Could you check a few things on this model? Use its own coordinates, in mm. Face numbers are marked on the shaded views. Round coordinates to 2 decimals unless told otherwise and drop trailing zeros. Loops run counter-clockwise (first coordinate to the right, second up) from the corner with the lowest first, then second, coordinate; pieces in that order, holes last. Notation, with made-up numbers: (85, -35.75) - (127, -35.75) arc R12 ccw to (127, -29.75) - close; hole circle Ø10 at (87.25, 57.25). An arc over 180 degrees is marked (long way). Answer as CSV lines item,"result". Start each with the question number.
1) I'm going to push flat-ended pins straight in: pin 1 Ø6 at (x, y) = (-373, 93) entering from +Z; pin 2 Ø2 at (x, y) = (-18.5, -324) entering from +Z. Where does each tip first touch, or does it pass through?
2) Please list where these lines run through material, in increasing order: line 1 along X through (y, z) = (324.2, 670); line 2 along Z through (x, y) = (488.8, 295); line 3 along Z through (x, y) = (474, -324.05).
3) Suppose I cut it at A-A, the plane z = 288. Write out the boundary of the cut face in (x, y).
4) Suppose I cut it at C-C, the plane x = -194. Write out the boundary of the cut face in (y, z), then the cut area to 3 significant figures.
5) We'd pull the mould along X, two halves only. Please class the marked faces 1, 2, 3 and 4: pulls with the +X half, pulls with the -X half, needs draft (parallel to the pull), parting line crosses it, or undercut.
6) Suppose I cut it at B-B, the plane y = -149. Write out the boundary of the cut face in (x, z).
```python
from build123d import *

# Parameters (mm, degrees)
EXTRUDE_1_DEPTH          = 325
EXTRUDE_2_DEPTH          = 2
EXTRUDE_3_DEPTH          = 2
SKETCH_5_W               = 30
SKETCH_5_H               = 650
EXTRUDE_4_DEPTH          = 2
SKETCH_6_R               = 4.5
CUT_EXTRUDE_1_DEPTH      = 10
CUT_EXTRUDE_2_DEPTH      = 1140
CUT_EXTRUDE_2_DEPTH_BACK = 345
SKETCH_7_R               = 4.5
SKETCH_8_R               = 4.5
CUT_EXTRUDE_3_DEPTH      = 10


with BuildPart() as part:
    # 草图1 → 凸台-拉伸1 (new, symmetric)
    with BuildSketch(Plane(origin=(0, 0, 0), x_dir=(1, 0, 0), z_dir=(0, 1, 0))):
        Polygon((-490, 700), (490, 700), (490, -700), (488, -700), (488, 698), (-488, 698), (-488, -700), (-490, -700), align=None)
    extrude(amount=EXTRUDE_1_DEPTH, both=True)

    # 草图2 → 凸台-拉伸2 (add)
    with BuildSketch(Plane(origin=(0, 325, 0), x_dir=(1, 0, 0), z_dir=(0, 1, 0))):
        Polygon((-490, 700), (-490, -700), (-460, -700), (-460, 670), (460, 670), (460, -700), (490, -700), (490, 700), align=None)
    extrude(amount=-EXTRUDE_2_DEPTH)

    # 草图3 → 凸台-拉伸3 (add)
    with BuildSketch(Plane.XZ.offset(325)):
        Polygon((490, -700), (490, 700), (460, 700), (460, -670), (-460, -670), (-460, 700), (-490, 700), (-490, -700), align=None)
    extrude(amount=-EXTRUDE_3_DEPTH)

    # 草图5 → 凸台-拉伸4 (add)
    with BuildSketch(Plane.XY.offset(700)):
        with Locations((-475, 0)):
            Rectangle(SKETCH_5_W, SKETCH_5_H)
    extrude(amount=-EXTRUDE_4_DEPTH)

    # 草图6 → 切除-拉伸1 (cut)
    with BuildSketch(Plane(origin=(0, 0, 698), x_dir=(-1, 0, 0), z_dir=(0, 0, -1))):
        with Locations((474, -246)):
            Circle(SKETCH_6_R)
        with Locations((474, -186)):
            Circle(SKETCH_6_R)
        with Locations((474, 295)):
            Circle(SKETCH_6_R)
        with Locations((474, 57)):
            Circle(SKETCH_6_R)
        with Locations((474, -23)):
            Circle(SKETCH_6_R)
        with Locations((474, -123)):
            Circle(SKETCH_6_R)
    extrude(amount=-CUT_EXTRUDE_1_DEPTH, mode=Mode.SUBTRACT)

    # 草图7 → 切除-拉伸2 (cut, two sides: drawn at the far end of the back side and taken through both)
    with BuildSketch(Plane.XZ.offset(-323).offset(-CUT_EXTRUDE_2_DEPTH_BACK)):
        with Locations(Location((-474, 670, 0), (0, 0, 90))):
            Circle(SKETCH_7_R)
        with Locations(Location((-474, 0, 0), (0, 0, 90))):
            Circle(SKETCH_7_R)
        with Locations(Location((-474, -684, 0), (0, 0, 90))):
            Circle(SKETCH_7_R)
        with Locations(Location((474, -684, 0), (0, 0, 90))):
            Circle(SKETCH_7_R)
        with Locations(Location((0, -684, 0), (0, 0, 90))):
            Circle(SKETCH_7_R)
        with Locations(Location((474, 0, 0), (0, 0, 90))):
            Circle(SKETCH_7_R)
        with Locations(Location((474, 670, 0), (0, 0, 90))):
            Circle(SKETCH_7_R)
    extrude(amount=CUT_EXTRUDE_2_DEPTH + CUT_EXTRUDE_2_DEPTH_BACK, mode=Mode.SUBTRACT)

    # 草图8 → 切除-拉伸3 (cut)
    with BuildSketch(Plane(origin=(490, 0, 0), x_dir=(0, 0, -1), z_dir=(1, 0, 0))):
        with Locations((-330, 295)):
            Circle(SKETCH_8_R)
        with Locations((-670, 295)):
            Circle(SKETCH_8_R)
        with Locations((-670, -295)):
            Circle(SKETCH_8_R)
        with Locations((-330, -295)):
            Circle(SKETCH_8_R)
        with Locations((-330, 0)):
            Circle(SKETCH_8_R)
        with Locations((-670, 0)):
            Circle(SKETCH_8_R)
    extrude(amount=-CUT_EXTRUDE_3_DEPTH, mode=Mode.SUBTRACT)


solid = part.part
```
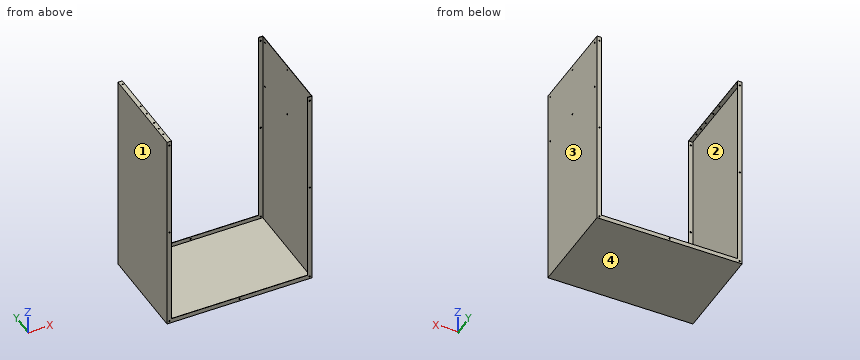
Filled sheet:
1,pin 1,"z = -698"
1,pin 2,"z = -670"
2,line 1,"-490 to -478.5, -469.5 to -460, 460 to 469.5, 478.5 to 490"
2,line 2,"-700 to 325.5, 334.5 to 665.5, 674.5 to 700"
2,line 3,"-700 to -688.5, -679.5 to -4.5, 4.5 to 665.5, 674.5 to 700"
3,outline,"(-490, -325) - (-460, -325) - (-460, -323) - (-488, -323) - (-488, 323) - (-460, 323) - (-460, 325) - (-490, 325) - close; (460, -325) - (490, -325) - (490, 325) - (460, 325) - (460, 323) - (488, 323) - (488, -323) - (460, -323) - close"
4,outline,"(-325, -700) - (325, -700) - (325, -670) - (323, -670) - (323, -698) - (-323, -698) - (-323, -670) - (-325, -670) - close"
4,area,"1,410 mm²"
5,face 1,"pulls with the -X half"
5,face 2,"undercut"
5,face 3,"pulls with the +X half"
5,face 4,"needs draft"
6,outline,"(-490, -700) - (490, -700) - (490, 700) - (488, 700) - (488, -698) - (-488, -698) - (-488, 698) - (-460, 698) - (-460, 700) - (-490, 700) - close"
